Verification items for the finished model (mm, model axes). Give positions to 0.01 mm unless a question says otherwise; leave off trailing zeros. Loops run counter-clockwise (first coordinate to the right, second up) from the corner with the lowest first, then second, coordinate; pieces in that order, holes last. Notation, with made-up numbers: (62.5, -34) -> (106.5, -34) arc R12 cw to (106.5, -17) -> close; hole circle Ø1 at (35, 5.5). An arc over 180 degrees is marked (long way). Answer in a Markdown table with one row per item. Add a question column.
Q1. Section check B-B on x = -25. Enter the section's corners in (y, z).
Q2. Release check for a two-part mould opening along X. For faces 1 (the face through (24.8, 0.5, -48.5)), 2 (the face through (-1, 0, -19)) record: pulls with the +X half, pulls with the -X half, needs draft (parallel to the pull), parting line crosses it, or undercut.
Q3. Section check D-D on z = -75.5. Enter the section's corners in (x, y).
Q4. Material ranges on probe 1 along X at (y, z) = (0.55, -75.5); probe 2 along X at (y, z) = (0.75, 32); probe 3 along X at (y, z) = (0.65, -29), recorded low to high.
Q5. Section check A-A on z = -3. Enter the section's corners in (x, y).
Q6. Section check C-C on y = 0.35. Enter the section's corners in (x, z), and give its area (3 significant figures).
```python
from build123d import *

# Parameters (mm, degrees)
SKETCH_1_W          = 100
SKETCH_1_H          = 165
EXTRUDE_1_DEPTH     = 1
SKETCH_2_R          = 2.5
CUT_EXTRUDE_1_DEPTH = 97.474089786


with BuildPart() as part:
    # 草图1 → 凸台-拉伸1 (new body)
    with BuildSketch(Plane(origin=(0, 0, 0), x_dir=(1, 0, 0), z_dir=(0, 1, 0))):
        Rectangle(SKETCH_1_W, SKETCH_1_H)
    extrude(amount=EXTRUDE_1_DEPTH)

    # 草图2 → 切除-拉伸1 (cut, through all)
    with BuildSketch(Plane(origin=(0, 1, 0), x_dir=(1, 0, 0), z_dir=(0, 1, 0))):
        with Locations(Location((-25, 75.5, 0), (0, 0, 270))):
            Circle(SKETCH_2_R)
        with Locations(Location((25, 75.5, 0), (0, 0, 270))):
            Circle(SKETCH_2_R)
        with BuildLine():
            Line((-36, -82.5), (-36, -12.5))
            ThreePointArc((-36, -12.5), (-25, -1.5), (-14, -12.5))
            Line((-14, -12.5), (-14, -82.5))
            ThreePointArc((-14, -82.5), (-25, -93.5), (-36, -82.5))
        make_face()
        with BuildLine():
            Line((14, -82.5), (14, 37.5))
            ThreePointArc((14, 37.5), (25, 48.5), (36, 37.5))
            Line((36, 37.5), (36, -82.5))
            ThreePointArc((36, -82.5), (25, -93.5), (14, -82.5))
        make_face()
    extrude(amount=-CUT_EXTRUDE_1_DEPTH, mode=Mode.SUBTRACT)


solid = part.part
```
Taken from the geometry:
| question | item | result |
|---|---|---|
| 1 | outline | (0, -82.5) -> (1, -82.5) -> (1, -78) -> (0, -78) -> close; (0, -73) -> (1, -73) -> (1, 1.5) -> (0, 1.5) -> close |
| 2 | face 1 | undercut |
| 2 | face 2 | needs draft |
| 3 | outline | (-50, 0) -> (-27.5, 0) -> (-27.5, 1) -> (-50, 1) -> close; (-22.5, 0) -> (22.5, 0) -> (22.5, 1) -> (-22.5, 1) -> close; (27.5, 0) -> (50, 0) -> (50, 1) -> (27.5, 1) -> close |
| 4 | probe 1 | x = -50 to -27.5, -22.5 to 22.5, 27.5 to 50 |
| 4 | probe 2 | x = -50 to -36, -14 to 14, 36 to 50 |
| 4 | probe 3 | x = -50 to 14, 36 to 50 |
| 5 | outline | (-50, 0) -> (14, 0) -> (14, 1) -> (-50, 1) -> close; (36, 0) -> (50, 0) -> (50, 1) -> (36, 1) -> close |
| 6 | outline | (-50, -82.5) -> (50, -82.5) -> (50, 82.5) -> (36, 82.5) -> (36, -37.5) arc R11 cw to (14, -37.5) -> (14, 82.5) -> (-14, 82.5) -> (-14, 12.5) arc R11 cw to (-36, 12.5) -> (-36, 82.5) -> (-50, 82.5) -> close; hole circle Ø5 at (-25, -75.5); hole circle Ø5 at (25, -75.5) |
| 6 | area | 11,900 mm² |
